Check sheet for the modelled part. Datum: model origin and axes. Units: mm. Face numbers are marked on the shaded views. Round coordinates to 2 decimals unless told otherwise and drop trailing zeros. Loops run counter-clockwise (first coordinate to the right, second up) from the corner with the lowest first, then second, coordinate; pieces in that order, holes last. Notation, with made-up numbers: (74.25, 33) -> (98.25, 33) arc R25 cw to (98.25, 52) -> close; hole circle Ø3 at (85, 6). An arc over 180 degrees is marked (long way). Return JSON: item names as keys, results as strings.
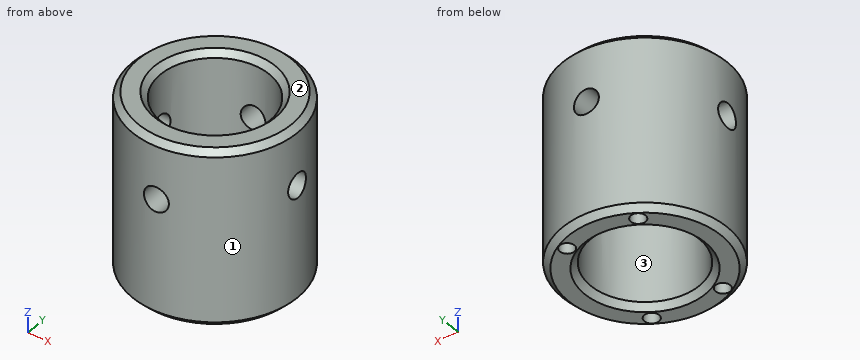
from build123d import *

# Parameters (mm, degrees)
SKETCH1_R             = 14
SKETCH1_R_2           = 9.25
BOSS_EXTRUDE1_DEPTH   = 15
SKETCH2_W             = 2.1
SKETCH2_H             = 14
SKETCH4_W             = 2.1
SKETCH4_H             = 14
M5_TAPPED_HOLE3_D     = 4.2
M5_TAPPED_HOLE4_D     = 4.2
M3_TAPPED_HOLE1_D     = 2.5
M3_TAPPED_HOLE1_DEPTH = 7.5
M3_TAPPED_HOLE1_TIP   = 0.751075774
CHAMFER1_SIZE         = 1


with BuildPart() as part:
    # Sketch1 → Boss-Extrude1 (new, symmetric)
    with BuildSketch(Plane.XY):
        Circle(SKETCH1_R)
        Circle(SKETCH1_R_2, mode=Mode.SUBTRACT)
    extrude(amount=BOSS_EXTRUDE1_DEPTH, both=True)

    # Sketch2 → M5 Tapped Hole1 (revolve, cut)
    with BuildSketch(Plane(origin=(0, 0, 5), x_dir=(0, 0, 1), z_dir=(1, 0, 0))):
        with Locations((1.05, 7)):
            Rectangle(SKETCH2_W, SKETCH2_H)
    revolve(axis=Axis((0, 6.35, 5), (0, -1, 0)), mode=Mode.SUBTRACT)

    # Sketch4 → M5 Tapped Hole2 (revolve, cut)
    with BuildSketch(Plane(origin=(0, 0, 5), x_dir=(0, 0, 1), z_dir=(0, 1, 0))):
        with Locations((1.05, 7)):
            Rectangle(SKETCH4_W, SKETCH4_H)
    revolve(axis=Axis((-6.35, 0, 5), (1, 0, 0)), mode=Mode.SUBTRACT)

    # M5 Tapped Hole3 (through all)
    with Locations(Plane.XZ):
        with Locations((0, 5)):
            Hole(M5_TAPPED_HOLE3_D / 2)

    # M5 Tapped Hole4 (through all)
    with Locations(Plane(origin=(0, 0, 0), x_dir=(0, 0, -1), z_dir=(1, 0, 0))):
        with Locations((-5, 0)):
            Hole(M5_TAPPED_HOLE4_D / 2)

    # M3 Tapped Hole1
    with Locations(Plane(origin=(0, 0, -15), x_dir=(-1, 0, 0), z_dir=(0, 0, -1))):
        with Locations((6, 10), (6, -10), (-6, -10), (-6, 10)):
            Hole(M3_TAPPED_HOLE1_D / 2, depth=M3_TAPPED_HOLE1_DEPTH)
            with Locations((0, 0, -(M3_TAPPED_HOLE1_DEPTH + M3_TAPPED_HOLE1_TIP / 2))):  # 118° drill point
                Cone(0, M3_TAPPED_HOLE1_D / 2, M3_TAPPED_HOLE1_TIP, mode=Mode.SUBTRACT)

    # Chamfer1
    chamfer1_edges = [part.edges().sort_by_distance(p)[0] for p in [
        (-14, 0, -15),
        (-14, 0, 15),
        (-9.25, 0, -15),
        (-9.25, 0, 15),
    ]]
    chamfer(chamfer1_edges, length=CHAMFER1_SIZE)


solid = part.part
Q1. Section check C-C (z = 5.5). Record the boundary of the cut face in (x, y), then the cut area to 3 significant figures.
Results list:
{"outline": "(-13.85, -2.04) arc R14 ccw to (-2.04, -13.85) -> (-2.04, -9.02) arc R9.25 cw to (-9.02, -2.04) -> close; (-13.85, 2.04) -> (-9.02, 2.04) arc R9.25 cw to (-2.04, 9.02) -> (-2.04, 13.85) arc R14 ccw to start; (2.04, -13.85) arc R14 ccw to (13.85, -2.04) -> (9.02, -2.04) arc R9.25 cw to (2.04, -9.02) -> close; (2.04, 9.02) arc R9.25 cw to (9.02, 2.04) -> (13.85, 2.04) arc R14 ccw to (2.04, 13.85) -> close", "area": "269 mm^2"}
Q2. Material ranges on line 1 (X direction, y = 10, z = -12.75); line 2 (X direction, y = -10.25, z = -10.5); line 3 (Z direction, x = -6, y = 10), recorded low to high.
Results list:
{"line 1": "-9.8 to -7.25, -4.75 to 4.75, 7.25 to 9.8", "line 2": "-9.54 to -7.22, -4.78 to 4.78, 7.22 to 9.54", "line 3": "-6.75 to 15"}
Q3. Draft check along X on the marked faces 1, 2 and 3. Enter one of: released by +X, released by -X, zero draft, split by the parting line, or undercut.
Results list:
{"face 1": "split by the parting line", "face 2": "zero draft", "face 3": "undercut"}
Q4. Section check D-D (z = -9). Record the boundary of the cut face in (x, y).
Results list:
{"outline": "circle Ø28 at (0, 0); hole circle Ø18.5 at (0, 0); hole circle Ø2.5 at (-6, -10); hole circle Ø2.5 at (-6, 10); hole circle Ø2.5 at (6, -10); hole circle Ø2.5 at (6, 10)"}
Q5. Section check A-A (x = 0). Record the boundary of the cut face in (y, z).
Results list:
{"outline": "(-14, -14) -> (-13, -15) -> (-10.25, -15) -> (-9.25, -14) -> (-9.25, 2.9) -> (-14, 2.9) -> close; (-14, 7.1) -> (-9.25, 7.1) -> (-9.25, 14) -> (-10.25, 15) -> (-13, 15) -> (-14, 14) -> close; (9.25, -14) -> (10.25, -15) -> (13, -15) -> (14, -14) -> (14, 2.9) -> (9.25, 2.9) -> close; (9.25, 7.1) -> (14, 7.1) -> (14, 14) -> (13, 15) -> (10.25, 15) -> (9.25, 14) -> close"}
Q6. Go/stop test with flat-tipped pins: pin 1 (5 mm diameter, centred on x = 1.5, y = -4, fed in from -Z); pin 2 (2 mm diameter, centred on x = -6, y = 10, fed in from -Z); pin 3 (3 mm diameter, centred on x = 3.5, z = 9.5, fed in from -Y); pin 4 (3 mm diameter, centred on x = -7, y = 5, fed in from -Z). Record where each tip stops, or that it passes through.
Results list:
{"pin 1": "through", "pin 2": "z = -7.35", "pin 3": "y = -13.86", "pin 4": "z = -14.85"}
